The listing builds one solid part. Answer for the finished solid, in the listing's coordinates (mm). Coordinates: 2 decimals unless noted, no trailing zeros. Loops run counter-clockwise (first coordinate to the right, second up) from the corner with the lowest first, then second, coordinate; pieces in that order, holes last. Notation, with made-up numbers: M 20.5,8.25 L 54.5,8.25 A29 cw 54.5,33.25 Z; hole C -16.5,41 d3. An arc over 180 degrees is marked long. Return JSON: item names as keys, results as strings. Group by question number.
1. Section A-A (y = -1.75) is taken. Write down the section's boundary in (x, z).
2. The mould has two halves that part along X. Classify faces 1 (the face through (5, 6, 5)), 2 (the face through (1.802, -0.084, 5.723)), 3 (the face through (-11.2, 0.1, -6.6)): pulls with the +X half, pulls with the -X half, needs draft (parallel to the pull), parting line crosses it, or undercut.
3. Section B-B (x = 0) is taken. Write down the section's boundary in (y, z), then the cut area to 3 significant figures.
4. Straight lines are drawn through the part: L1, parallel to Z at x = 2, y = 4; L2, parallel to Z at x = 2.5, y = -3; L3, parallel to X at y = 3.5, z = 3.75. For each, find the intervals that lie inside material, in ascending order. Write a range as from..to.
5. Given P1, Ø3, axis at y = -0.5, z = 10.5, coming from the +X side; P2, Ø1, axis at y = -4, z = -7.5, coming from the +X side; P3, Ø2, axis at x = 5.5, y = -4.5, coming from the -Z side, each flat-ended and moving along its own axis, determine where each tip first touches the part or whether it passes through.
```python
from build123d import *

# Parameters (mm, degrees)
HEX_NUT_PROFILE_R                     = 6
HEX_NUT_BODY_DEPTH                    = 6
CHAMFER_CIRCLE_23_OUTSIDE_W           = 98.006
CHAMFER_CIRCLE_23_OUTSIDE_H           = 93.984
CHAMFER_CIRCLE_23_OUTSIDE_R           = 11.5
CORNER_CHAMFER_50_DEPTH               = 24.202011407
CORNER_CHAMFER_50_DRAFT               = -50
CORNER_CHAMFER_MIRROR_COPY_1_SKETCH_W = 98.006
CORNER_CHAMFER_MIRROR_COPY_1_SKETCH_H = 93.984
CORNER_CHAMFER_MIRROR_COPY_1_SKETCH_R = 11.5
CORNER_CHAMFER_MIRROR_COPY_1_DEPTH    = 24.202011407
CORNER_CHAMFER_MIRROR_COPY_1_DRAFT    = -50


with BuildPart() as part:
    # Hex Nut Profile → Hex Nut Body (new, symmetric)
    with BuildSketch(Plane(origin=(0, 0, 0), x_dir=(1, 0, 0), z_dir=(0, 1, 0))):
        Polygon((15.011106999, 0), (7.505553499, 13), (-7.505553499, 13), (-15.011106999, 0), (-7.505553499, -13), (7.505553499, -13), align=None)
        with Locations(Location((0, 0, 0), (0, 0, 270))):
            Circle(HEX_NUT_PROFILE_R, mode=Mode.SUBTRACT)
    extrude(amount=HEX_NUT_BODY_DEPTH, both=True)


with BuildPart() as corner_chamfer_50_tool:
    # Chamfer Circle Ø23 outside → Corner Chamfer 50° (with draft: the straight prism first)
    with BuildSketch(Plane(origin=(0, 6, 0), x_dir=(1, 0, 0), z_dir=(0, 1, 0))):
        Rectangle(CHAMFER_CIRCLE_23_OUTSIDE_W, CHAMFER_CIRCLE_23_OUTSIDE_H)
        Circle(CHAMFER_CIRCLE_23_OUTSIDE_R, mode=Mode.SUBTRACT)
    extrude(amount=-CORNER_CHAMFER_50_DEPTH)
    # Corner Chamfer 50°: the draft: its side faces are tilted about the plane it starts from
    corner_chamfer_50_sides = [corner_chamfer_50_tool.faces().sort_by_distance(p)[0] for p in [
        (0, -6.101005704, 46.992),
        (49.003, -6.101005704, 0),
        (0, -6.101005704, -46.992),
        (-49.003, -6.101005704, 0),
        (-11.5, -6.101005704, 0),
    ]]
    draft(corner_chamfer_50_sides, Plane(origin=(0, 6, 0), x_dir=(1, 0, 0), z_dir=(0, 1, 0)), CORNER_CHAMFER_50_DRAFT)


with BuildPart() as part_1:
    add(part.part)

    # Corner Chamfer 50°: cut by corner_chamfer_50_tool
    add(corner_chamfer_50_tool.part, mode=Mode.SUBTRACT)


with BuildPart() as corner_chamfer_mirror_copy_1_tool:
    # Corner Chamfer Mirror copy 1 sketch → Corner Chamfer Mirror copy 1 (with draft: the straight prism first)
    with BuildSketch(Plane.XZ.offset(6)):
        Rectangle(CORNER_CHAMFER_MIRROR_COPY_1_SKETCH_W, CORNER_CHAMFER_MIRROR_COPY_1_SKETCH_H)
        Circle(CORNER_CHAMFER_MIRROR_COPY_1_SKETCH_R, mode=Mode.SUBTRACT)
    extrude(amount=-CORNER_CHAMFER_MIRROR_COPY_1_DEPTH)
    # Corner Chamfer Mirror copy 1: the draft: its side faces are tilted about the plane it starts from
    corner_chamfer_mirror_copy_1_sides = [corner_chamfer_mirror_copy_1_tool.faces().sort_by_distance(p)[0] for p in [
        (0, 6.101005704, 46.992),
        (49.003, 6.101005704, 0),
        (0, 6.101005704, -46.992),
        (-49.003, 6.101005704, 0),
        (-11.5, 6.101005704, 0),
    ]]
    draft(corner_chamfer_mirror_copy_1_sides, Plane.XZ.offset(6), CORNER_CHAMFER_MIRROR_COPY_1_DRAFT)


with BuildPart() as part_2:
    add(part_1.part)

    # Corner Chamfer Mirror copy 1: cut by corner_chamfer_mirror_copy_1_tool
    add(corner_chamfer_mirror_copy_1_tool.part, mode=Mode.SUBTRACT)


solid = part_2.part
```
Worked out:
{
 "1": {"outline": "M -15.01,0 L -7.51,-13 L 7.51,-13 L 15.01,0 L 7.51,13 L -7.51,13 Z; hole C 0,0 d12"},
 "2": {"face 1": "needs draft", "face 2": "undercut", "face 3": "pulls with the -X half"},
 "3": {"outline": "M -6,-11.5 L -4.74,-13 L 4.74,-13 L 6,-11.5 L 6,-6 L -6,-6 Z; M -6,6 L 6,6 L 6,11.5 L 4.74,13 L -4.74,13 L -6,11.5 Z", "area": "164 mm^2"},
 "4": {"L1": "-13..-5.66, 5.66..13", "L2": "-13..-5.45, 5.45..13", "L3": "-12.85..-4.68, 4.68..12.85"},
 "5": {"P1": "x = 9.81", "P2": "x = 10.97", "P3": "z = -13"}
}
